```python
from build123d import *

# Parameters (mm, degrees)
SKETCH_1_R      = 1.025
SKETCH_1_R_2    = 1.3
SKETCH_1_R_3    = 1.55
EXTRUDE_1_DEPTH = 1.5
FILLET_R2_1_R   = 2


with BuildPart() as part:
    # 草图1 → 凸台-拉伸1 (new body)
    with BuildSketch(Plane(origin=(0, 0, 0), x_dir=(0, 0, -1), z_dir=(1, 0, 0))):
        with BuildLine():
            Line((-9.25, 0), (-9.25, 19.75))
            Line((-9.25, 19.75), (-19.25, 19.75))
            Line((-19.25, 19.75), (-19.25, 0))
            ThreePointArc((-19.25, 0), (-20.641242789, -3.358757211), (-24, -4.75))
            Line((-24, -4.75), (-25.4, -4.75))
            Line((-25.4, -4.75), (-25.4, -14.75))
            Line((-25.4, -14.75), (-24, -14.75))
            ThreePointArc((-24, -14.75), (-13.570174977, -10.429825023), (-9.25, 0))
        make_face()
        with Locations((-11.438131953, -2.182194118)):
            Circle(SKETCH_1_R, mode=Mode.SUBTRACT)
        with Locations((-13.411740816, -7.102905565)):
            Circle(SKETCH_1_R, mode=Mode.SUBTRACT)
        with Locations((-17.216155884, -10.795460111)):
            Circle(SKETCH_1_R, mode=Mode.SUBTRACT)
        with Locations((-22.193559229, -12.621381531)):
            Circle(SKETCH_1_R, mode=Mode.SUBTRACT)
        with Locations((-11.25, 3.116215025)):
            Circle(SKETCH_1_R, mode=Mode.SUBTRACT)
        with Locations((-21.4, -7.034912935)):
            Circle(SKETCH_1_R_2, mode=Mode.SUBTRACT)
        with Locations((-16.917350474, -2.466997302)):
            Circle(SKETCH_1_R_3, mode=Mode.SUBTRACT)
        with Locations((-16.75, 5.25)):
            Circle(SKETCH_1_R_3, mode=Mode.SUBTRACT)
        with Locations((-13, 15.75)):
            Circle(SKETCH_1_R_3, mode=Mode.SUBTRACT)
        with Locations((-16.5, 11.05)):
            Circle(SKETCH_1_R_2, mode=Mode.SUBTRACT)
    extrude(amount=EXTRUDE_1_DEPTH)

    # R2 圆角1
    fillet_r2_1_edges = [part.edges().sort_by_distance(p)[0] for p in [
        (0.75, 19.75, 19.25),
        (0.75, 19.75, 9.25),
        (0.75, -4.75, 25.4),
        (0.75, -14.75, 25.4),
    ]]
    fillet(fillet_r2_1_edges, radius=FILLET_R2_1_R)


solid = part.part
```
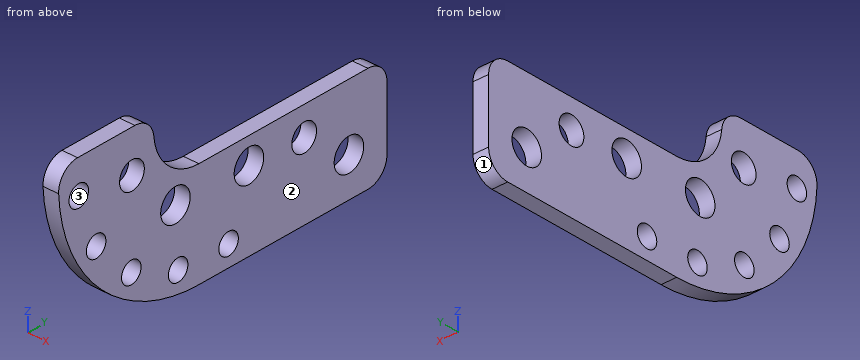
Verification items for the finished model (mm, model axes). Face numbers are marked on the shaded views. Round coordinates to 2 decimals unless told otherwise and drop trailing zeros. Order: outer loops, then holes, each group sorted by start corner. A loop starts at its lowest first (then second) coordinate and runs counter-clockwise, first axis right, second up.
1) Draft check along Z on the marked faces 1, 2 and 3. Enter one of: +Z half, -Z half, draft (parallel to the pull), parting line (faces both ways), or undercut.
Geometry says:
face 1: -Z half
face 2: draft
face 3: undercut
2) Cross-section at B-B, the plane y = 15.75. Record the cut outline in (x, z).
Geometry says:
outline: (0, 9.25) - (1.5, 9.25) - (1.5, 11.45) - (0, 11.45) - close; (0, 14.55) - (1.5, 14.55) - (1.5, 19.25) - (0, 19.25) - close
3) Cross-section at D-D, the plane z = 13. Record the cut outline in (x, y), plus the area to 3 significant figures.
Geometry says:
outline: (0, -9.83) - (1.5, -9.83) - (1.5, -8.04) - (0, -8.04) - close; (0, -6.16) - (1.5, -6.16) - (1.5, 14.2) - (0, 14.2) - close; (0, 17.3) - (1.5, 17.3) - (1.5, 19.75) - (0, 19.75) - close
area: 36.9 mm2
4) Material ranges on line 1 (Y direction, x = 1.2, z = 12.5); line 2 (Y direction, x = 0.65, z = 18) (3 decimals); line 3 (Y direction, x = 0.5, z = 12), recorded low to high.
Geometry says:
line 1: y = -9.24 to -7.57, -6.63 to 14.28, 17.22 to 19.75
line 2: y = -13.475 to -11.456, -10.135 to -3.576, -1.358 to 4.333, 6.167 to 19.604
line 3: y = -8.58 to -3.04, -1.32 to 2.42, 3.81 to 14.57, 16.93 to 19.75
5) Depth check by flat-ended pin: pin 1 (3.5 mm diameter, centred on y = -7.03, z = 21.4, fed in from +X). Enter the tip coordinate at first touch or a pass-through.
Geometry says:
pin 1: stops at x = 1.5
6) Cross-section at A-A, the plane z = 16.5. Record the cut outline in (x, y), plus the area to 3 significant figures.
Geometry says:
outline: (0, -12.7) - (1.5, -12.7) - (1.5, -11.53) - (0, -11.53) - close; (0, -10.06) - (1.5, -10.06) - (1.5, -3.96) - (0, -3.96) - close; (0, -0.97) - (1.5, -0.97) - (1.5, 3.72) - (0, 3.72) - close; (0, 6.78) - (1.5, 6.78) - (1.5, 9.75) - (0, 9.75) - close; (0, 12.35) - (1.5, 12.35) - (1.5, 19.75) - (0, 19.75) - close
area: 33.5 mm2
7) Cross-section at C-C, the plane z = 20.5. Record the cut outline in (x, y).
Geometry says:
outline: (0, -14.33) - (1.5, -14.33) - (1.5, -7.97) - (0, -7.97) - close; (0, -6.1) - (1.5, -6.1) - (1.5, -3.21) - (0, -3.21) - close
